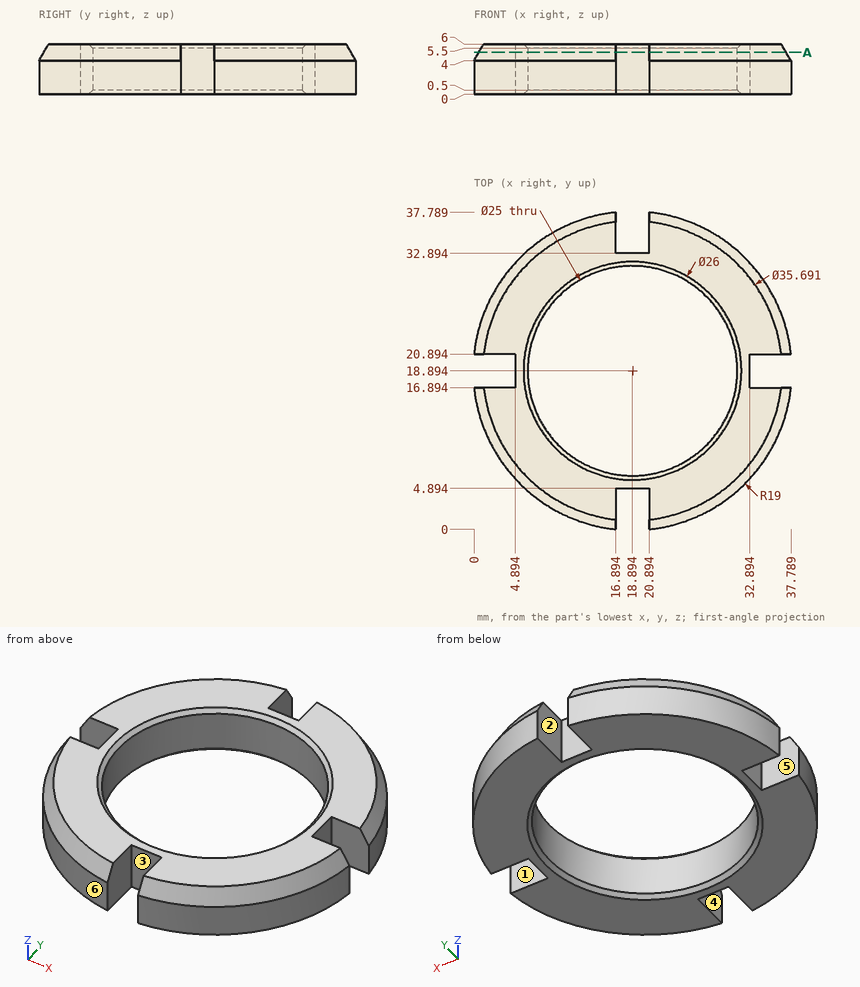
Geometry check sheet. Reference: drawing and pictorial views, mm from the part's lowest x, y, z. A direction names the side the tool comes from. Coordinates: 2 decimals unless noted, no trailing zeros. Order: outer loops, then holes, each group sorted by start corner. A loop starts at its lowest first (then second) coordinate and runs counter-clockwise, first axis right, second up. Notation, with made-up numbers: M -6,22 L 11,22 A16 ccw 11,50 Z; hole C 63,-23.75 d4. An arc over 180 degrees is marked long. Return JSON: item names as keys, results as strings.
1) Cross-section at A-A, the plane z = 5. Record the boundary of the cut face in (x, y) (1 decimal), and give its area (3 significant figures).
Answer list:
{"outline": "M 0.6,16.9 A18.4 ccw 16.9,0.6 L 16.9,4.9 L 20.9,4.9 L 20.9,0.6 A18.4 ccw 37.2,16.9 L 32.9,16.9 L 32.9,20.9 L 37.2,20.9 A18.4 ccw 20.9,37.2 L 20.9,32.9 L 16.9,32.9 L 16.9,37.2 A18.4 ccw 0.6,20.9 L 4.9,20.9 L 4.9,16.9 Z; hole C 18.9,18.9 d25", "area": "505 mm2"}
2) Access from +Z, -Z, +X, -X, +Y, -Y to the whole of each face (thin tool, end or side, straight path). Record for the marked faces 1, 2 and 3.
Answer list:
{"face 1": "+Z, -Z, +X", "face 2": "+Z, -Z, +Y", "face 3": "+Z, -Z, -Y"}
3) Thickness scan on L1, parallel to X at y = 19, z = 2.75 (1 decimal); L2, parallel to X at y = 24.5, z = 1.75; L3, parallel to Y at x = 25, z = 3.75 (1 decimal). Record the ranges inside material, lowest first. Write a range as [from, to].
Answer list:
{"L1": "[4.9, 6.4], [31.4, 32.9]", "L2": "[0.74, 7.72], [30.07, 37.05]", "L3": "[0.9, 8], [29.8, 36.9]"}
4) Release check for a two-part mould opening along X. For the marked faces 4, 5 and 6 record: +X half, -X half, draft (parallel to the pull), parting line (faces both ways), or undercut.
Answer list:
{"face 4": "undercut", "face 5": "draft", "face 6": "-X half"}
5) Gauge pin test, flat ends, axial feed: pin 1 (1.5 mm diameter, centred on x = 34, z = 2, fed in from -Y); pin 2 (2 mm diameter, centred on y = 18, z = 3.5, fed in from -X); pin 3 (3 mm diameter, centred on x = 18.5, z = 3.5, fed in from -Y); pin 4 (3 mm diameter, centred on x = 18, z = 4.5, fed in from +Y). Record the tip position at first contact, or that the pin passes through.
Answer list:
{"pin 1": "y = 6.45", "pin 2": "x = 4.89", "pin 3": "y = 4.89", "pin 4": "y = 37.79"}
